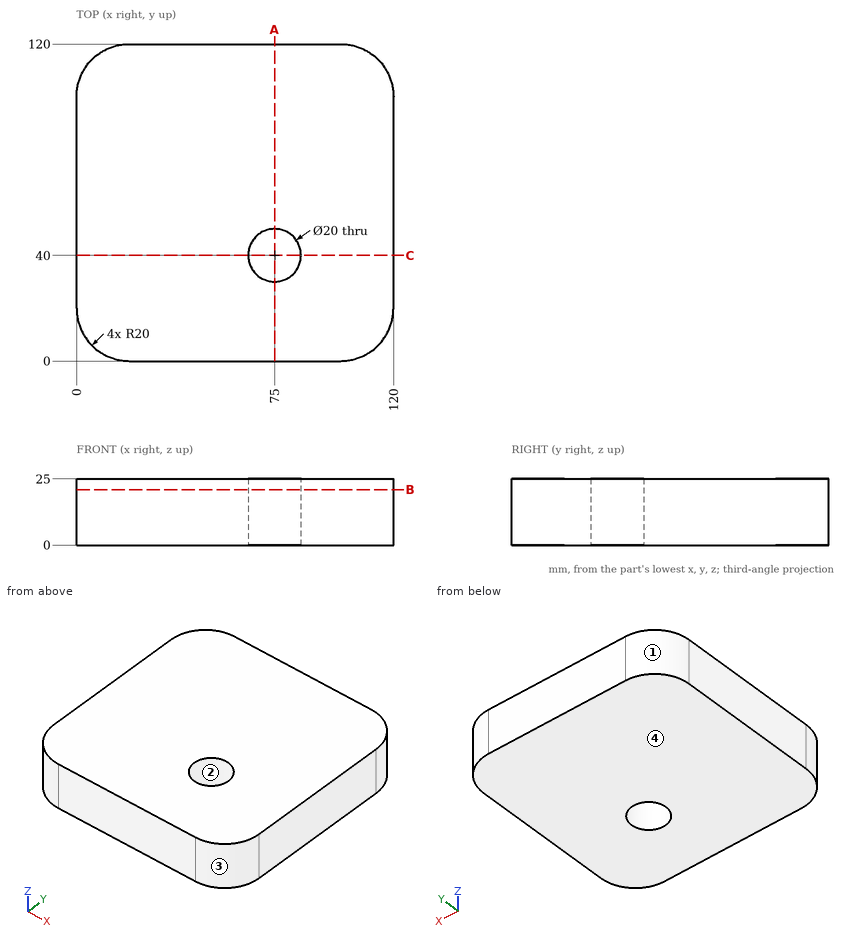
Here's the drawing with two shaded views (mm, measured from the low corner). I have some questions. Coordinates: 2 decimals unless noted, no trailing zeros. Write each loop counter-clockwise with the first axis right and the second up, starting at its lowest first coordinate (ties: lowest second). Pieces come first, ordered by that corner, then holes. Notation, with made-up numbers: M -2.5,-7.5 L 46.5,-7.5 A29 cw 46.5,29.5 Z; hole C 23.5,2 d10. An arc over 180 degrees is marked long. Answer as CSV lines item,"result". Start each with the question number.
1) I want a section at C-C, the plane y = 40. Please give me the cut outline in (x, z).
2) I want a section at A-A, the plane x = 75. Please give me the cut outline in (y, z).
3) I want a section at B-B, the plane z = 21. Please give me the cut outline in (x, y), and give its area (3 significant figures).
4) Please list where these lines run through material, in increasing order: line 1 (Y direction, x = 75, z = 7.75); line 2 (X direction, y = 48, z = 10.5); line 3 (X direction, y = 42, z = 22.75). Write a range as from..to.
5) We'd pull the mould along X, two halves only. Please class the marked faces 1, 2, 3 and 4: +X half, -X half, draft (parallel to the pull), parting line (faces both ways), or undercut.
Data:
1,outline,"M 0,0 L 65,0 L 65,25 L 0,25 Z; M 85,0 L 120,0 L 120,25 L 85,25 Z"
2,outline,"M 0,0 L 30,0 L 30,25 L 0,25 Z; M 50,0 L 120,0 L 120,25 L 50,25 Z"
3,outline,"M 0,20 A20 ccw 20,0 L 100,0 A20 ccw 120,20 L 120,100 A20 ccw 100,120 L 20,120 A20 ccw 0,100 Z; hole C 75,40 d20"
3,area,"13,700 mm^2"
4,line 1,"y = 0..30, 50..120"
4,line 2,"x = 0..69, 81..120"
4,line 3,"x = 0..65.2, 84.8..120"
5,face 1,"-X half"
5,face 2,"undercut"
5,face 3,"+X half"
5,face 4,"draft"
